Work out the finished part from the listing and answer in its coordinate system (mm). A direction names the side the tool comes from. Round coordinates to 2 decimals unless told otherwise and drop trailing zeros. Write each loop counter-clockwise with the first axis right and the second up, starting at its lowest first coordinate (ties: lowest second). Pieces come first, ordered by that corner, then holes.
1. Find section A-A (z = 0). Write down the section's boundary in (x, y).
2. Find section D-D (x = -8.25). Write down the section's boundary in (y, z).
3. Find section B-B (x = -3.75). Write down the section's boundary in (y, z).
4. Determine the mould class of faces 1 (the face through (7, 3, 0)), 2 (the face through (12, 0, 0)), 3 (the face through (-4, -2, -2.25)), 4 (the face through (-4, 1, 3)) for opening direction X: pulls with the +X half, pulls with the -X half, needs draft (parallel to the pull), parting line crosses it, or undercut.
5. Straight lines are drawn through the part: probe 1 along Z at (x, y) = (-5, -1); probe 2 along Y at (x, z) = (-9.75, -2.5); probe 3 along X at (y, z) = (3.5, -5.5). For each, find the intervals that lie inside material, in ascending order.
6. A flat-ended cylindrical pin translates along its axis: pin 1 Ø4 at (y, z) = (3.5, 5.5) entering from -X. Find the tip coordinate at first contact, or state that the pin passes through.
7. A tool of negligible diameter and unlimited length cuts with its end or side. For faces 5 (the face through (-4, -2, 2.25)), 6 (the face through (-12, -2, 0)), from which of +Z, -Z, +X, -X, +Y, -Y can it reach the whole face along a straight path? Write none if from no direction.
8. Find section C-C (y = 0). Write down the section's boundary in (x, z).
```python
from build123d import *

# Parameters (mm, degrees)
BOSS_EXTRUDE1_DEPTH = 7.5
CUT_EXTRUDE1_REACH  = 17.37


with BuildPart() as part:
    # Sketch1 → Boss-Extrude1 (new, symmetric)
    with BuildSketch(Plane.XY):
        Polygon((4, 1), (-12, 1), (-12, -5), (12, -5), (12, 5), (10, 5), align=None)
    extrude(amount=BOSS_EXTRUDE1_DEPTH, both=True)

    # Sketch2 → Cut-Extrude1 (cut, up to next)
    with BuildSketch(Plane(origin=(0, 1, 0), x_dir=(1, 0, 0), z_dir=(0, 1, 0)), mode=Mode.PRIVATE) as cut_extrude1_sk1:
        with BuildLine():
            Line((-7, 2.25), (-1, 2.25))
            ThreePointArc((-1, 2.25), (1.25, 0), (-1, -2.25))
            Line((-1, -2.25), (-7, -2.25))
            ThreePointArc((-7, -2.25), (-9.25, 0), (-7, 2.25))
        make_face()
    cut_extrude1_tool1 = extrude(cut_extrude1_sk1.sketch, amount=-CUT_EXTRUDE1_REACH, mode=Mode.PRIVATE) & part.part
    add(cut_extrude1_tool1.solids().sort_by_distance((-4, 1, 0))[0], mode=Mode.SUBTRACT)


solid = part.part
```
Worked answers:
1. outline: (-12, -5) - (-9.25, -5) - (-9.25, 1) - (-12, 1) - close; (1.25, -5) - (12, -5) - (12, 5) - (10, 5) - (4, 1) - (1.25, 1) - close
2. outline: (-5, -7.5) - (1, -7.5) - (1, -1.87) - (-5, -1.87) - close; (-5, 1.87) - (1, 1.87) - (1, 7.5) - (-5, 7.5) - close
3. outline: (-5, -7.5) - (1, -7.5) - (1, -2.25) - (-5, -2.25) - close; (-5, 2.25) - (1, 2.25) - (1, 7.5) - (-5, 7.5) - close
4. face 1: pulls with the -X half
4. face 2: pulls with the +X half
4. face 3: undercut
4. face 4: needs draft
5. probe 1: z = -7.5 to -2.25, 2.25 to 7.5
5. probe 2: y = -5 to 1
5. probe 3: x = 7.75 to 12
6. pin 1: stops at x = 4.75
7. face 5: +Y, -Y
7. face 6: +Z, -Z, -X, +Y, -Y
8. outline: (-12, -7.5) - (12, -7.5) - (12, 7.5) - (-12, 7.5) - close; hole (-7, -2.25) - (-1, -2.25) arc R2.25 ccw to (-1, 2.25) - (-7, 2.25) arc R2.25 ccw to start
